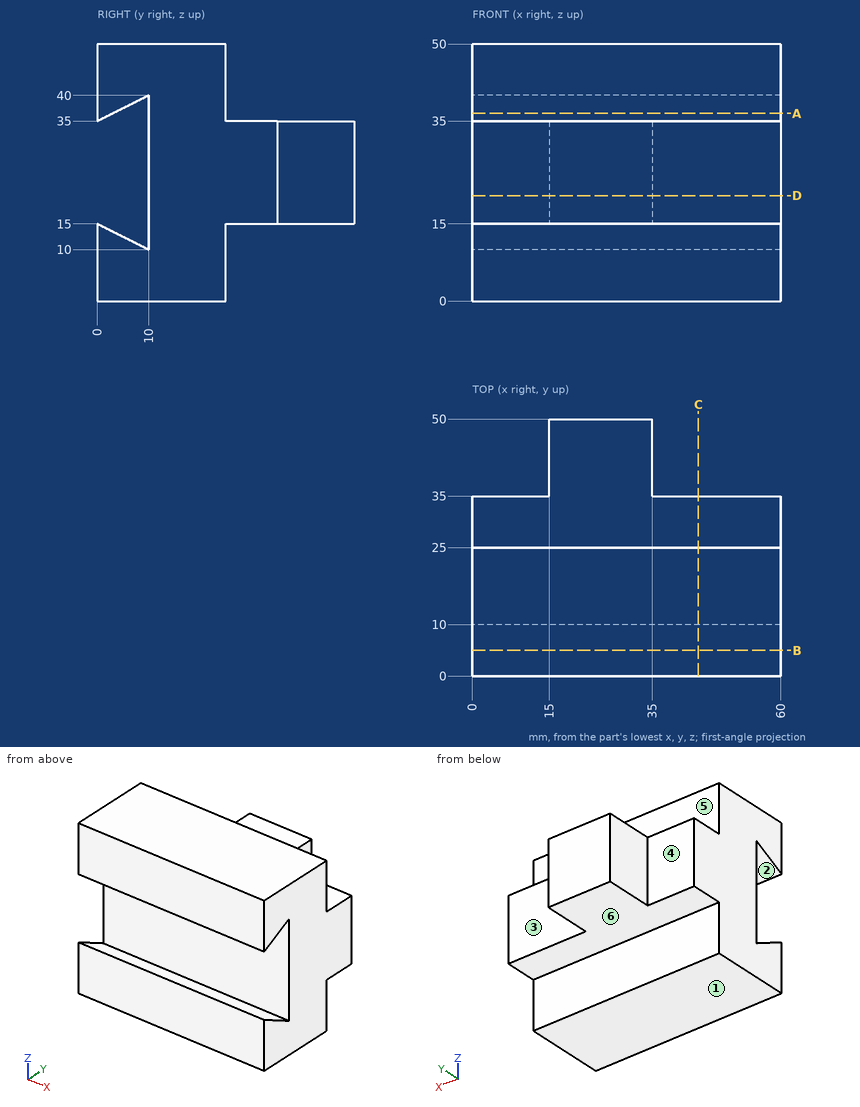
Verification items for this drawing (mm, ordinates from the low corner). A direction names the side the tool comes from. Give positions to 0.01 mm unless a question says otherwise; leave off trailing zeros. Loops run counter-clockwise (first coordinate to the right, second up) from the corner with the lowest first, then second, coordinate; pieces in that order, holes last. Notation, with made-up numbers: M 30,1.5 L 50,1.5 A17 cw 50,31.5 Z; hole C -35.5,-28.5 d10. An arc over 180 degrees is marked long. Write each question's results on one line, items separated by ' | '.
1) Tool access check on the marked faces 4, 5 and 6. Record the directions out of +Z, -Z, +X, -X, +Y, -Y that give a thin tool (end or side, any length) a straight path to the whole face; none if there is none.
Answers follow:
face 4: +Z, -Z, -X, +Y | face 5: +Z, +X, -X, +Y | face 6: -Z, +X, -X, +Y
2) Section check C-C, the plane x = 44. Record the boundary of the cut face in (y, z), plus the area to 3 significant figures.
Answers follow:
outline: M 0,0 L 25,0 L 25,15 L 35,15 L 35,35 L 25,35 L 25,50 L 0,50 L 0,35 L 10,40 L 10,10 L 0,15 Z | area: 1,200 mm2
3) Section check D-D, the plane z = 20.5. Record the boundary of the cut face in (x, y).
Answers follow:
outline: M 0,10 L 60,10 L 60,35 L 35,35 L 35,50 L 15,50 L 15,35 L 0,35 Z
4) Thickness scan on line 1 (Z direction, x = 29, y = 33.5); line 2 (Y direction, x = 25, z = 16.5); line 3 (Y direction, x = 25.5, z = 13.5). Record the ranges inside material, lowest first.
Answers follow:
line 1: 15 to 35 | line 2: 10 to 50 | line 3: 0 to 3, 10 to 25
5) Gauge pin test, flat ends, axial feed: pin 1 (4.5 mm diameter, centred on x = 41.5, z = 8.5, fed in from +Y); pin 2 (12 mm diameter, centred on y = 40.5, z = 22.5, fed in from -X); pin 3 (4 mm diameter, centred on y = 6.5, z = 17, fed in from +X); pin 4 (20 mm diameter, centred on x = 29.5, y = 37, fed in from +Z). Record the tip position at first contact, or that the pin passes through.
Answers follow:
pin 1: y = 25 | pin 2: x = 0 | pin 3: through | pin 4: z = 35
6) Section check B-B, the plane y = 5. Record the boundary of the cut face in (x, z).
Answers follow:
outline: M 0,0 L 60,0 L 60,12.5 L 0,12.5 Z; M 0,37.5 L 60,37.5 L 60,50 L 0,50 Z
7) Section check A-A, the plane z = 36.5. Record the boundary of the cut face in (x, y).
Answers follow:
outline: M 0,0 L 60,0 L 60,3 L 0,3 Z; M 0,10 L 60,10 L 60,25 L 0,25 Z
8) Release check for a two-part mould opening along Z. For the marked faces 1, 2 and 3 record: +Z half, -Z half, draft (parallel to the pull), parting line (faces both ways), or undercut.
Answers follow:
face 1: -Z half | face 2: undercut | face 3: draft
